Can you work these out from the model? Positions are in its coordinate system, mm. A direction names the side the tool comes from. Give positions to 0.01 mm unless a question says otherwise; leave off trailing zeros. Order: outer loops, then holes, each group sorted by start corner. A loop starts at its lowest first (then second) coordinate and runs counter-clockwise, first axis right, second up. Notation, with made-up numbers: (-23.75, 11.5) - (35.25, 11.5) arc R30 cw to (35.25, 35.5) - close; hole circle Ø4 at (70, 55.25). An arc over 180 degrees is marked (long way). Answer as CSV lines item,"result".
```python
from build123d import *

# Parameters (mm, degrees)
SKETCH_1_W                = 52
SKETCH_1_H                = 16
EXTRUDE_1_DEPTH           = 10
HOLE_WIZARD_1_D           = 3.4
HOLE_WIZARD_1_DEPTH       = 38
HOLE_WIZARD_1_CBORE_D     = 6
HOLE_WIZARD_1_CBORE_DEPTH = 3.4
HOLE_WIZARD_1_TIP         = 1.021463052
CHAMFER_1_SIZE            = 5
CHAMFER_1_SIZE2           = 2.886751346
CHAMFER_2_SIZE            = 5
CHAMFER_2_SIZE2           = 2.886751346


with BuildPart() as part:
    # 草图1 → 凸台-拉伸1 (new body)
    with BuildSketch(Plane.XY):
        Rectangle(SKETCH_1_W, SKETCH_1_H)
    extrude(amount=EXTRUDE_1_DEPTH)

    # 打孔尺寸(%根据)内六角圆柱头螺钉的类型1
    with Locations(Plane(origin=(0, 0, 0), x_dir=(-1, 0, 0), z_dir=(0, 0, -1))):
        with Locations((-17, 0), (17, 0)):
            CounterBoreHole(HOLE_WIZARD_1_D / 2, HOLE_WIZARD_1_CBORE_D / 2, HOLE_WIZARD_1_CBORE_DEPTH, depth=HOLE_WIZARD_1_DEPTH)
            with Locations((0, 0, -(HOLE_WIZARD_1_DEPTH + HOLE_WIZARD_1_TIP / 2))):  # 118° drill point
                Cone(0, HOLE_WIZARD_1_D / 2, HOLE_WIZARD_1_TIP, mode=Mode.SUBTRACT)

    # 倒角1
    chamfer_1_edges = [part.edges().sort_by_distance(p)[0] for p in [
        (26, 0, 0),
    ]]
    chamfer_1_side = [part.faces().sort_by_distance(p)[0] for p in [
        (0, 0, 0),
    ]]
    chamfer(chamfer_1_edges, length=CHAMFER_1_SIZE, length2=CHAMFER_1_SIZE2, reference=chamfer_1_side[0])

    # 倒角2
    chamfer_2_edges = [part.edges().sort_by_distance(p)[0] for p in [
        (-26, 0, 0),
    ]]
    chamfer_2_side = [part.faces().sort_by_distance(p)[0] for p in [
        (-2.703280464, 0, 0),
    ]]
    chamfer(chamfer_2_edges, length=CHAMFER_2_SIZE, length2=CHAMFER_2_SIZE2, reference=chamfer_2_side[0])


solid = part.part
```
1) I want a section at D-D on y = 4. Write out the boundary of the cut face in (x, z).
Answer block:
outline,"(-26, 2.89) - (-21, 0) - (21, 0) - (26, 2.89) - (26, 10) - (-26, 10) - close"
2) I need wall thicknesses on line 1 along Y through (x, z) = (17, 6); line 2 along Z through (x, y) = (17, 2); line 3 along Y through (x, z) = (17, 1.85). Which ranges of each line are inside material? Lowest first, please. Write a range as [from, to].
Answer block:
line 1,"[-8, -1.7], [1.7, 8]"
line 2,"[3.4, 10]"
line 3,"[-8, -3], [3, 8]"
3) I want a section at B-B on y = 0. Write out the boundary of the cut face in (x, z).
Answer block:
outline,"(-26, 2.89) - (-21, 0) - (-20, 0) - (-20, 3.4) - (-18.7, 3.4) - (-18.7, 10) - (-26, 10) - close; (-15.3, 3.4) - (-14, 3.4) - (-14, 0) - (14, 0) - (14, 3.4) - (15.3, 3.4) - (15.3, 10) - (-15.3, 10) - close; (18.7, 3.4) - (20, 3.4) - (20, 0) - (21, 0) - (26, 2.89) - (26, 10) - (18.7, 10) - close"
4) If we mould it in two halves opening along X, with no side actions, what happens to faces 1 (the cylindrical face through (-15.38, 0.51, 6.75)), 2 (the flat face through (-26, 0, 6)), 3 (the flat face through (0, 8, 5))? For each: +X half, -X half, draft (parallel to the pull), parting line (faces both ways), or undercut.
Answer block:
face 1,"undercut"
face 2,"-X half"
face 3,"draft"
5) I want a section at A-A on x = 17. Write out the boundary of the cut face in (y, z).
Answer block:
outline,"(-8, 0) - (-3, 0) - (-3, 3.4) - (-1.7, 3.4) - (-1.7, 10) - (-8, 10) - close; (1.7, 3.4) - (3, 3.4) - (3, 0) - (8, 0) - (8, 10) - (1.7, 10) - close"
6) I want a section at C-C on z = 8.75. Write out the boundary of the cut face in (x, y), plus the area to 3 significant figures.
Answer block:
outline,"(-26, -8) - (26, -8) - (26, 8) - (-26, 8) - close; hole circle Ø3.4 at (-17, 0); hole circle Ø3.4 at (17, 0)"
area,"814 mm2"
7) I'm going to push a flat-ended pin straight in: P1, Ø3, axis at x = 17, y = -1, coming from the -Z side. Where does the tip first touch, or does it pass through?
Answer block:
P1,"z = 3.4"
8) Which directions (+Z, -Z, +X, -X, +Y, -Y) give clear straight access to the entire face, cutting with the end or side of a thin tool? Please do faces 4 (the cylindrical face through (20, 0, 2)), 5 (the flat face through (0, 0, 0)).
Answer block:
face 4,"-Z"
face 5,"-Z, +X, -X, +Y, -Y"
